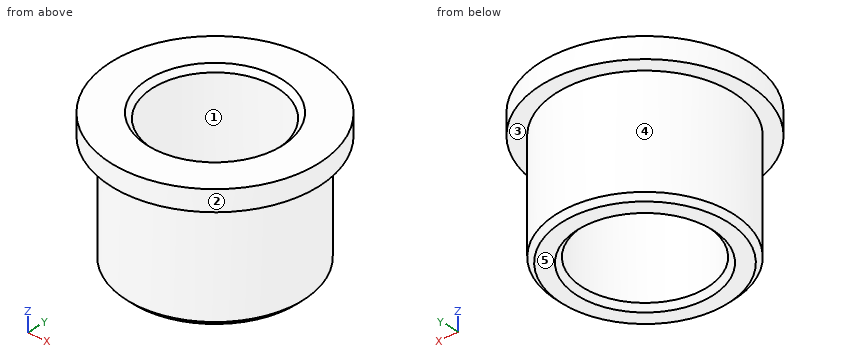
from build123d import *

# Parameters (mm, degrees)
SKETCH1_R           = 8.5
BOSS_EXTRUDE1_DEPTH = 13
SKETCH2_R           = 10
BOSS_EXTRUDE2_DEPTH = 2
SKETCH3_R           = 6
CUT_EXTRUDE1_DEPTH  = 25
CHAMFER1_SIZE       = 0.5


with BuildPart() as part:
    # Sketch1 → Boss-Extrude1 (new body)
    with BuildSketch(Plane.XY):
        with Locations(Location((0, 0, 0), (0, 0, 180))):
            Circle(SKETCH1_R)
    extrude(amount=BOSS_EXTRUDE1_DEPTH)

    # Sketch2 → Boss-Extrude2 (add)
    with BuildSketch(Plane.XY.offset(13)):
        Circle(SKETCH2_R)
    extrude(amount=-BOSS_EXTRUDE2_DEPTH)

    # Sketch3 → Cut-Extrude1 (cut)
    with BuildSketch(Plane(origin=(0, 0, 0), x_dir=(-1, 0, 0), z_dir=(0, 0, -1))):
        Circle(SKETCH3_R)
    extrude(amount=-CUT_EXTRUDE1_DEPTH, mode=Mode.SUBTRACT)

    # Chamfer1
    chamfer1_edges = [part.edges().sort_by_distance(p)[0] for p in [
        (6, 0, 13),
        (6, 0, 0),
        (8.5, 0, 0),
    ]]
    chamfer(chamfer1_edges, length=CHAMFER1_SIZE)


solid = part.part
CAD build for the part. Positions are in the model's coordinates, mm. Face numbers are marked on the shaded views. A direction names the side the tool comes from. Coordinates: 2 decimals unless noted, no trailing zeros. Write each loop counter-clockwise with the first axis right and the second up, starting at its lowest first coordinate (ties: lowest second). Pieces come first, ordered by that corner, then holes. Notation, with made-up numbers: (-33.5, -7.75) - (7.5, -7.75) arc R17 cw to (7.5, 17.25) - close; hole circle Ø11 at (13, 13.25). An arc over 180 degrees is marked (long way). Use a Markdown table: item, result. Add a question column.
Item 1: Band-saw the part on D-D, the plane z = 11.75. Give the cut face in (x, y).
Item 2: Band-saw the part on A-A, the plane y = 0. Give the cut face in (x, z).
Item 3: Band-saw the part on C-C, the plane z = 9.75. Give the cut face in (x, y).
Item 4: Mould opens along X. For the marked faces 1, 2 and 3 say: pulls with the +X half, pulls with the -X half, needs draft (parallel to the pull), parting line crosses it, or undercut.
Item 5: Flat gauge pins, fed straight in: pin 1 (1.5 mm diameter, centred on x = 5.5, z = 11, fed in from -Y); pin 2 (6 mm diameter, centred on x = 4, z = 9, fed in from -Y); pin 3 (3 mm diameter, centred on x = 7, z = 4.5, fed in from -Y). Where does each tip first touch, or does it go through?
Item 6: 3-axis set-ups, long thin cutter, end or side, ignore diameter. For the marked faces 4 and 5: which of +Z, -Z, +X, -X, +Y, -Y reach the whole face in a straight line?
Item 7: Drill centre lines: L1, parallel to Y at x = 0, z = 9.25; L2, parallel to X at y = -4, z = 11.25; L3, parallel to Y at x = -4.5, z = 7.25. Where is each one in solid material? Low to high. Write a range as from..to.
Numbers:
| question | item | result |
|---|---|---|
| 1 | outline | circle Ø20 at (0, 0); hole circle Ø12 at (0, 0) |
| 2 | outline | (-10, 11) - (-8.5, 11) - (-8.5, 0.5) - (-8, 0) - (-6.5, 0) - (-6, 0.5) - (-6, 12.5) - (-6.5, 13) - (-10, 13) - close; (6, 0.5) - (6.5, 0) - (8, 0) - (8.5, 0.5) - (8.5, 11) - (10, 11) - (10, 13) - (6.5, 13) - (6, 12.5) - close |
| 3 | outline | circle Ø17 at (0, 0); hole circle Ø12 at (0, 0) |
| 4 | face 1 | undercut |
| 4 | face 2 | parting line crosses it |
| 4 | face 3 | needs draft |
| 5 | pin 1 | y = -8.8 |
| 5 | pin 2 | y = -9.84 |
| 5 | pin 3 | y = -6.48 |
| 6 | face 4 | -Z |
| 6 | face 5 | -Z, +X, -X, +Y, -Y |
| 7 | L1 | -8.5..-6, 6..8.5 |
| 7 | L2 | -9.17..-4.47, 4.47..9.17 |
| 7 | L3 | -7.21..-3.97, 3.97..7.21 |
